Design review of the part built by this model. Coordinates are the model's own, in mm. A direction names the side the tool comes from. Coordinates: 2 decimals unless noted, no trailing zeros. Loops run counter-clockwise (first coordinate to the right, second up) from the corner with the lowest first, then second, coordinate; pieces in that order, holes last. Notation, with made-up numbers: (62.25, 6) -> (71.25, 6) arc R24 cw to (71.25, 27) -> close; hole circle Ø5 at (-2, 27.5). An arc over 180 degrees is marked (long way). Answer as a JSON object with one key per item and string values.
```python
from build123d import *

# Parameters (mm, degrees)
EXTRUDE_THIN1_DEPTH = 100
CUT_EXTRUDE1_DEPTH  = 79


with BuildPart() as part:
    # Sketch2 → Extrude-Thin1 (new, symmetric)
    with BuildSketch(Plane.XY.offset(-180)):
        Polygon((-191.015662361, 220), (-191.015662361, -100), (-103.254276677, -100), (-103.254276677, -90), (-181.015662361, -90), (-181.015662361, 220), align=None)
    extrude(amount=EXTRUDE_THIN1_DEPTH, both=True)

    # Sketch3 → Cut-Extrude1 (cut)
    with BuildSketch(Plane.XZ.offset(100)):
        Polygon((-139.911519959, -240), (-169.911519959, -180), (-139.911519959, -120), (-109.911519959, -180), align=None)
    extrude(amount=-CUT_EXTRUDE1_DEPTH, mode=Mode.SUBTRACT)


solid = part.part
```
1) Add section A-A, the plane z = -187. Give the boundary of the cut face in (x, y), and give its area (3 significant figures).
Completed:
{"outline": "(-191.02, -100) -> (-166.41, -100) -> (-166.41, -90) -> (-181.02, -90) -> (-181.02, 220) -> (-191.02, 220) -> close; (-113.41, -100) -> (-103.25, -100) -> (-103.25, -90) -> (-113.41, -90) -> close", "area": "3,450 mm²"}
2) Add section D-D, the plane y = 114. Give the boundary of the cut face in (x, z), and give its area (3 significant figures).
Completed:
{"outline": "(-191.02, -280) -> (-181.02, -280) -> (-181.02, -80) -> (-191.02, -80) -> close", "area": "2,000 mm²"}
3) Add section C-C, the plane z = -158.5. Give the boundary of the cut face in (x, y), and give its area (3 significant figures).
Completed:
{"outline": "(-191.02, -100) -> (-159.16, -100) -> (-159.16, -90) -> (-181.02, -90) -> (-181.02, 220) -> (-191.02, 220) -> close; (-120.66, -100) -> (-103.25, -100) -> (-103.25, -90) -> (-120.66, -90) -> close", "area": "3,590 mm²"}
4) For faces 5 (the flat face through (-125.12, -95.07, -149.58)), 6 (the flat face through (-159, -90, -156)), 7 (the flat face through (-177, -100, -179)), list the 3-axis set-ups (+Z, -Z, +X, -X, +Y, -Y) from which the entire face can be reached by the end or side of a thin tool; tool diameter is ignored.
Completed:
{"face 5": "+Y, -Y", "face 6": "+Z, -Z, +X, +Y", "face 7": "+Z, -Z, +X, -X, -Y"}
5) Wall thickness on probe 1 along X at (y, z) = (44.5, -173); probe 2 along Y at (x, z) = (-158, -129): over which ranges is each line inside the solid? List them lowest first.
Completed:
{"probe 1": "-191.02 to -181.02", "probe 2": "-100 to -90"}
6) Add section B-B, the plane x = -148. Give the boundary of the cut face in (y, z), and give its area (3 significant figures).
Completed:
{"outline": "(-100, -280) -> (-90, -280) -> (-90, -223.82) -> (-100, -223.82) -> close; (-100, -136.18) -> (-90, -136.18) -> (-90, -80) -> (-100, -80) -> close", "area": "1,120 mm²"}
7) The part is to be moulded in two halves that separate along X. For faces 1 (the flat face through (-191.016, 62, -179)), 2 (the flat face through (-155.12, -95.07, -150.42)), 3 (the flat face through (-103.254, -95, -179)), 4 (the flat face through (-183, 25, -80)), say which applies: pulls with the +X half, pulls with the -X half, needs draft (parallel to the pull), parting line crosses it, or undercut.
Completed:
{"face 1": "pulls with the -X half", "face 2": "undercut", "face 3": "pulls with the +X half", "face 4": "needs draft"}
